from build123d import *

# Parameters (mm, degrees)
SPOKE_WINDOWS_4X_DEPTH = 20


with BuildPart() as part:
    # Handwheel Profile Sketch → Handwheel Body (revolve)
    with BuildSketch(Plane.XY):
        with BuildLine():
            Line((-8, -37), (-17.5, -37))
            Line((-17.5, -37), (-17.5, -25.041311123))
            ThreePointArc((-17.5, -25.041311123), (-17.726042647, -24.117690362), (-18.353075311, -23.402847282))
            Line((-18.353075311, -23.402847282), (-36.983519773, -10.361536159))
            ThreePointArc((-36.983519773, -10.361536159), (-37.529165692, -10.092524223), (-38.130444462, -10))
            Line((-38.130444462, -10), (-47.5, -10))
            ThreePointArc((-47.5, -10), (-54.571067812, 7.071067812), (-37.5, 0))
            Line((-37.5, 0), (-16, -20))
            Line((-16, -20), (-4.2, -20))
            Line((-4.2, -20), (-4.2, -29))
            Line((-4.2, -29), (-8, -29))
            Line((-8, -29), (-8, -37))
        make_face()
    revolve(axis=Axis((0, 48.530715578, 0), (0, -1, 0)))

    # Spoke Windows Sketch → Spoke Windows 4x (cut)
    with BuildSketch(Plane(origin=(0, -20, 0), x_dir=(1, 0, 0), z_dir=(0, 1, 0))):
        with BuildLine():
            Line((19.364916731, 5), (34.641016151, 5))
            ThreePointArc((34.641016151, 5), (24.748737342, 24.748737342), (5, 34.641016151))
            Line((5, 34.641016151), (5, 19.364916731))
            ThreePointArc((5, 19.364916731), (14.142135624, 14.142135624), (19.364916731, 5))
        make_face()
        with BuildLine():
            Line((34.641016151, -5), (19.364916731, -5))
            ThreePointArc((19.364916731, -5), (14.142135624, -14.142135624), (5, -19.364916731))
            Line((5, -19.364916731), (5, -34.641016151))
            ThreePointArc((5, -34.641016151), (24.748737342, -24.748737342), (34.641016151, -5))
        make_face()
        with BuildLine():
            ThreePointArc((-5, 34.641016151), (-24.748737342, 24.748737342), (-34.641016151, 5))
            Line((-34.641016151, 5), (-19.364916731, 5))
            ThreePointArc((-19.364916731, 5), (-14.142135624, 14.142135624), (-5, 19.364916731))
            Line((-5, 19.364916731), (-5, 34.641016151))
        make_face()
        with BuildLine():
            ThreePointArc((-34.641016151, -5), (-24.748737342, -24.748737342), (-5, -34.641016151))
            Line((-5, -34.641016151), (-5, -19.364916731))
            ThreePointArc((-5, -19.364916731), (-14.142135624, -14.142135624), (-19.364916731, -5))
            Line((-19.364916731, -5), (-34.641016151, -5))
        make_face()
    extrude(amount=SPOKE_WINDOWS_4X_DEPTH, mode=Mode.SUBTRACT)


solid = part.part
Source: CAD feature listing. Evaluate the final solid. Frame: model axes, mm. A direction names the side the tool comes from. Coordinates: 2 decimals unless noted, no trailing zeros. Loops run counter-clockwise (first coordinate to the right, second up) from the corner with the lowest first, then second, coordinate; pieces in that order, holes last. Notation, with made-up numbers: (-17, -31) -> (41, -31) arc R7 cw to (41, -23) -> close; hole circle Ø2 at (0, -16). An arc over 180 degrees is marked (long way). Answer in a Markdown table with one row per item. Add a question column.
Q1. Section C-C on y = -14. Return the cut outline in (x, z).
Q2. Ray query, line 1 along Z through (x, y) = (0, -32); line 2 along Z through (x, y) = (0, -25). Return the intervals inside material, ascending.
Q3. Section B-B on z = 0. Return the cut outline in (x, y), and give its area (3 significant figures).
Q4. Section A-A on x = 0. Return the cut outline in (y, z), and give its area (3 significant figures).
Q5. Contact query for flat-ended pins moving along their axis: pin 1 Ø5.5 at (x, z) = (12, -16.5) entering from +Y; pin 2 Ø17 at (y, z) = (-10, -29) entering from -X; pin 3 Ø2 at (y, z) = (-13, -23) entering from +X. Output: stop coordinate, or through.
Q6. Reachability of faces 5 (the face through (-14.247, -18.166, -14.036)), 6 (the face through (-29, -13, -5)), 7 (the face through (0, -10, -39)) from +Z, -Z, +X, -X, +Y, -Y: full face, straight path, thin tool, end or side. Return the list, or none.
Q7. Pull-direction query (Z, two-part tool) for faces 1 (the face through (14.036, -18.166, -14.247)), 2 (the face through (-14.036, -18.166, 14.247)), 3 (the face through (5, -13, 29)), 4 (the face through (-24.525, -7.104, -24.97)); classes: pulls with the +Z half, pulls with the -Z half, needs draft (parallel to the pull), parting line crosses it, or undercut.
Q8. Section D-D on y = -27. Return the cut outline in (x, z), and give its area (3 significant figures).
Computed values:
| question | item | result |
|---|---|---|
| 1 | outline | (-31.39, -5) -> (-21.89, -5) arc R22.45 cw to (-21.89, 5) -> (-31.39, 5) arc R31.79 ccw to start; (-5, -31.39) arc R31.79 ccw to (5, -31.39) -> (5, -21.89) arc R22.45 cw to (-5, -21.89) -> close; (-5, 21.89) arc R22.45 cw to (5, 21.89) -> (5, 31.39) arc R31.79 ccw to (-5, 31.39) -> close; (21.89, -5) -> (31.39, -5) arc R31.79 ccw to (31.39, 5) -> (21.89, 5) arc R22.45 cw to start |
| 2 | line 1 | z = -17.5 to -8, 8 to 17.5 |
| 2 | line 2 | z = -17.5 to -4.2, 4.2 to 17.5 |
| 3 | outline | (-47.5, -10) -> (-38.13, -10) arc R2 cw to (-36.98, -10.36) -> (-18.35, -23.4) arc R2 cw to (-17.5, -25.04) -> (-17.5, -37) -> (-8, -37) -> (-8, -29) -> (-4.2, -29) -> (-4.2, -20) -> (-16, -20) -> (-37.5, 0) arc R10 ccw (long way) to start; (4.2, -29) -> (8, -29) -> (8, -37) -> (17.5, -37) -> (17.5, -25.04) arc R2 cw to (18.35, -23.4) -> (36.98, -10.36) arc R2 cw to (38.13, -10) -> (47.5, -10) arc R10 ccw (long way) to (37.5, 0) -> (16, -20) -> (4.2, -20) -> close |
| 3 | area | 1,370 mm^2 |
| 4 | outline | (-37, -17.5) -> (-25.04, -17.5) arc R2 cw to (-23.4, -18.35) -> (-10.36, -36.98) arc R2 cw to (-10, -38.13) -> (-10, -47.5) arc R10 ccw (long way) to (0, -37.5) -> (-20, -16) -> (-20, -4.2) -> (-29, -4.2) -> (-29, -8) -> (-37, -8) -> close; (-37, 8) -> (-29, 8) -> (-29, 4.2) -> (-20, 4.2) -> (-20, 16) -> (0, 37.5) arc R10 ccw (long way) to (-10, 47.5) -> (-10, 38.13) arc R2 cw to (-10.36, 36.98) -> (-23.4, 18.35) arc R2 cw to (-25.04, 17.5) -> (-37, 17.5) -> close |
| 4 | area | 1,370 mm^2 |
| 5 | pin 1 | stops at y = -16.28 |
| 5 | pin 2 | stops at x = -51.8 |
| 5 | pin 3 | stops at x = 5 |
| 6 | face 5 | -Z, -X, +Y |
| 6 | face 6 | +Y |
| 6 | face 7 | -Y |
| 7 | face 1 | pulls with the -Z half |
| 7 | face 2 | pulls with the +Z half |
| 7 | face 3 | undercut |
| 7 | face 4 | undercut |
| 8 | outline | circle Ø35 at (0, 0); hole circle Ø8.4 at (0, 0) |
| 8 | area | 907 mm^2 |
